Check sheet for the modelled part. Datum: model origin and axes. Units: mm. Coordinates: 2 decimals unless noted, no trailing zeros. Loops run counter-clockwise (first coordinate to the right, second up) from the corner with the lowest first, then second, coordinate; pieces in that order, holes last. Notation, with made-up numbers: M -4,57 L 4,57 A17 ccw 4,70 Z; hole C 28,-36 d7. An arc over 180 degrees is marked long. Return JSON: item names as keys, results as strings.
from build123d import *

# Parameters (mm, degrees)
SKETCH1_W           = 115
SKETCH1_H           = 128
BOSS_EXTRUDE1_DEPTH = 4
F_10_HOLE1_D        = 10
FILLET1_R           = 10
CUT_EXTRUDE1_REACH  = 88.407
SKETCH4_R           = 23


with BuildPart() as part:
    # Sketch1 → Boss-Extrude1 (new, symmetric)
    with BuildSketch(Plane.XY):
        Rectangle(SKETCH1_W, SKETCH1_H)
    extrude(amount=BOSS_EXTRUDE1_DEPTH, both=True)

    # Ø10 Hole1 (through all)
    with Locations(Plane.XY.offset(4)):
        with Locations((-34.926406871, 55.5), (49.926406871, 55.5), (49.926406871, -29.352813742), (-34.926406871, -29.352813742)):
            Hole(F_10_HOLE1_D / 2)

    # Fillet1
    fillet1_edges = [part.edges().sort_by_distance(p)[0] for p in [
        (57.5, -64, 0),
        (-57.5, -64, 0),
    ]]
    fillet(fillet1_edges, radius=FILLET1_R)

    # Sketch4 → Cut-Extrude1 (cut, up to next)
    with BuildSketch(Plane.XY.offset(4), mode=Mode.PRIVATE) as cut_extrude1_sk1:
        with Locations((7.5, 33.073593129)):
            Circle(SKETCH4_R)
    cut_extrude1_tool1 = extrude(cut_extrude1_sk1.sketch, amount=-CUT_EXTRUDE1_REACH, mode=Mode.PRIVATE) & part.part
    add(cut_extrude1_tool1.solids().sort_by_distance((7.5, 33.073593, 4))[0], mode=Mode.SUBTRACT)


solid = part.part
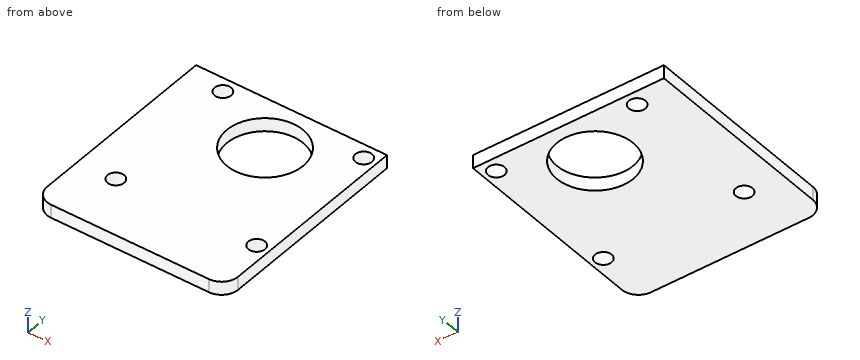
1) Section check A-A on x = 7.5. Record the cut outline in (y, z), then the cut area to 3 significant figures.
Answers:
{"outline": "M -64,-4 L 10.07,-4 L 10.07,4 L -64,4 Z; M 56.07,-4 L 64,-4 L 64,4 L 56.07,4 Z", "area": "656 mm²"}
2) Section check C-C on x = -38. Record the cut outline in (y, z), then the cut area to 3 significant figures.
Answers:
{"outline": "M -64,-4 L -33.3,-4 L -33.3,4 L -64,4 Z; M -25.41,-4 L 51.56,-4 L 51.56,4 L -25.41,4 Z; M 59.44,-4 L 64,-4 L 64,4 L 59.44,4 Z", "area": "898 mm²"}
3) Scan lines: line 1 along Y through (x, z) = (7.5, 0.75); line 2 along Y through (x, z) = (-30.5, 1.5); line 3 along X through (y, z) = (39.5, 0.5). Record each from-to range of solid material in increasing order. Write a range as [from, to].
Answers:
{"line 1": "[-64, 10.07], [56.07, 64]", "line 2": "[-64, -31.68], [-27.03, 53.17], [57.83, 64]", "line 3": "[-57.5, -14.58], [29.58, 57.5]"}
4) Section check D-D on y = 53.5. Record the cut outline in (x, z).
Answers:
{"outline": "M -57.5,-4 L -39.51,-4 L -39.51,4 L -57.5,4 Z; M -30.34,-4 L -3.07,-4 L -3.07,4 L -30.34,4 Z; M 18.07,-4 L 45.34,-4 L 45.34,4 L 18.07,4 Z; M 54.51,-4 L 57.5,-4 L 57.5,4 L 54.51,4 Z"}
5) Section check B-B on y = 18.5. Record the cut outline in (x, z).
Answers:
{"outline": "M -57.5,-4 L -10.29,-4 L -10.29,4 L -57.5,4 Z; M 25.29,-4 L 57.5,-4 L 57.5,4 L 25.29,4 Z"}
